The listing builds one solid part. Answer for the finished solid, in the listing's coordinates (mm). A direction names the side the tool comes from. Give positions to 0.01 mm unless a question says otherwise; leave off trailing zeros. Loops run counter-clockwise (first coordinate to the right, second up) from the corner with the lowest first, then second, coordinate; pieces in that order, holes last.
Item 1: A tool of negligible diameter and unlimited length cuts with its end or side. For faces 1 (the face through (26.503, -5.07, 6.631)), 2 (the face through (10, -32, 6)), from which of +Z, -Z, +X, -X, +Y, -Y can it reach the whole face along a straight path? Write none if from no direction.
Item 2: Consider line 1 along Y through (x, z) = (6.25, 6); line 2 along X through (y, z) = (-6, 5.75); line 3 along Y through (x, z) = (2.75, 6). Determine where each line is inside the solid, lowest interval first.
Item 3: Section B-B, the plane y = -22.5 is taken. Give the vertices of the cut face in (x, z).
Item 4: Section C-C, the plane x = 24.5 is taken. Give the vertices of the cut face in (y, z).
Item 5: Section A-A, the plane z = 6 is taken. Give the vertices of the cut face in (x, y), and give its area (3 significant figures).
Item 6: Section D-D, the plane y = -8.5 is taken. Give the vertices of the cut face in (x, z), and give its area (3 significant figures).
Item 7: Each of these flat-tipped pins is pushed along its axis until it touches: pin 1 Ø2 at (y, z) = (-16, 3.5) entering from +X; pin 2 Ø3.5 at (x, z) = (52.5, 6) entering from +Y; pin 3 Ø3.5 at (x, z) = (40.5, 8.5) entering from -Y. Where does it stop, or does it pass through?
Item 8: The mould has two halves that part along Z. Classify faces 3 (the face through (4.93, -39.773, 5.642)), 4 (the face through (5, -50, 6)), 5 (the face through (21, -6, 0)): pulls with the +Z half, pulls with the -Z half, needs draft (parallel to the pull), parting line crosses it, or undercut.
from build123d import *

# Parameters (mm, degrees)
BOSS_EXTRUDE1_DEPTH   = 12
M5_TAPPED_HOLE1_D     = 4.2
M5_TAPPED_HOLE1_DEPTH = 12.4
M5_TAPPED_HOLE1_TIP   = 1.2618073
M5_CLEARANCE_HOLE1_D  = 5.5
CHAMFER2_SIZE         = 1
FILLET1_R             = 5


with BuildPart() as part:
    # Sketch1 → Boss-Extrude1 (new body)
    with BuildSketch(Plane.XY):
        Polygon((3, 0), (60, 0), (60, -10), (10, -10), (10, -50), (0, -50), (0, -3), align=None)
    extrude(amount=BOSS_EXTRUDE1_DEPTH)

    # M5 Tapped Hole1
    with Locations(Plane(origin=(0, 0, 0), x_dir=(-1, 0, 0), z_dir=(0, 1, 0))):
        with Locations((-52.5, 6), (-24.5, 6)):
            Hole(M5_TAPPED_HOLE1_D / 2, depth=M5_TAPPED_HOLE1_DEPTH)
            with Locations((0, 0, -(M5_TAPPED_HOLE1_DEPTH + M5_TAPPED_HOLE1_TIP / 2))):  # 118° drill point
                Cone(0, M5_TAPPED_HOLE1_D / 2, M5_TAPPED_HOLE1_TIP, mode=Mode.SUBTRACT)

    # M5 Clearance Hole1 (through all)
    with Locations(Plane(origin=(10, 0, 0), x_dir=(0, 0, -1), z_dir=(1, 0, 0))):
        with Locations((-6, -42.5), (-6, -22.5)):
            Hole(M5_CLEARANCE_HOLE1_D / 2)

    # Chamfer2
    chamfer2_edges = [part.edges().sort_by_distance(p)[0] for p in [
        (60, -5, 0),
        (5, -50, 12),
        (60, -5, 12),
        (5, -50, 0),
    ]]
    chamfer(chamfer2_edges, length=CHAMFER2_SIZE)

    # Fillet1
    fillet1_edges = [part.edges().sort_by_distance(p)[0] for p in [
        (10, -10, 6),
    ]]
    fillet(fillet1_edges, radius=FILLET1_R)


solid = part.part
Worked answers:
1. face 1: +Y, -Y
1. face 2: +Z, -Z, +X, -Y
2. line 1: y = -50 to -45.25, -39.75 to -25.25, -19.75 to 0
2. line 2: x = 0 to 22.41, 26.59 to 50.41, 54.59 to 60
2. line 3: y = -50 to -45.25, -39.75 to -25.25, -19.75 to -0.25
3. outline: (0, 0) - (10, 0) - (10, 3.25) - (0, 3.25) - close; (0, 8.75) - (10, 8.75) - (10, 12) - (0, 12) - close
4. outline: (-10, 0) - (0, 0) - (0, 3.9) - (-10, 3.9) - close; (-10, 8.1) - (0, 8.1) - (0, 12) - (-10, 12) - close
5. outline: (0, -50) - (10, -50) - (10, -45.25) - (0, -45.25) - close; (0, -39.75) - (10, -39.75) - (10, -25.25) - (0, -25.25) - close; (0, -19.75) - (10, -19.75) - (10, -15) arc R5 cw to (15, -10) - (22.4, -10) - (22.4, 0) - (3, 0) - (0, -3) - close; (26.6, -10) - (50.4, -10) - (50.4, 0) - (26.6, 0) - close; (54.6, -10) - (60, -10) - (60, 0) - (54.6, 0) - close
5. area: 807 mm2
6. outline: (0, 0) - (59, 0) - (60, 1) - (60, 11) - (59, 12) - (0, 12) - close; hole circle Ø4.2 at (24.5, 6); hole circle Ø4.2 at (52.5, 6)
6. area: 691 mm2
7. pin 1: stops at x = 10
7. pin 2: passes through
7. pin 3: stops at y = -10
8. face 3: undercut
8. face 4: needs draft
8. face 5: pulls with the -Z half
